```python
from build123d import *

# Parameters (mm, degrees)
SKETCH1_R           = 5
BOSS_EXTRUDE1_DEPTH = 5


with BuildPart() as part:
    # Sketch1 → Boss-Extrude1 (new body)
    with BuildSketch(Plane.XY):
        with BuildLine():
            Line((9.797958971, 5), (150.202041029, 5))
            ThreePointArc((150.202041029, 5), (152.091863394, 5.370899501), (153.70131209, 6.428571429))
            ThreePointArc((153.70131209, 6.428571429), (169, 0), (153.70131209, -6.428571429))
            ThreePointArc((153.70131209, -6.428571429), (152.091863394, -5.370899501), (150.202041029, -5))
            Line((150.202041029, -5), (9.797958971, -5))
            ThreePointArc((9.797958971, -5), (7.908136606, -5.370899501), (6.29868791, -6.428571429))
            ThreePointArc((6.29868791, -6.428571429), (-9, 0), (6.29868791, 6.428571429))
            ThreePointArc((6.29868791, 6.428571429), (7.908136606, 5.370899501), (9.797958971, 5))
        make_face()
        Circle(SKETCH1_R, mode=Mode.SUBTRACT)
        with Locations((160, 0)):
            Circle(SKETCH1_R, mode=Mode.SUBTRACT)
    extrude(amount=BOSS_EXTRUDE1_DEPTH)


solid = part.part
```
The listing builds one solid part. Answer for the finished solid, in the listing's coordinates (mm). A direction names the side the tool comes from. Round coordinates to 2 decimals unless told otherwise and drop trailing zeros. Loops run counter-clockwise (first coordinate to the right, second up) from the corner with the lowest first, then second, coordinate; pieces in that order, holes last.
Q1. For a pull along Y with two mould halves and no side action, classify faces 1 (the face through (7.93, -5.36, 2.46)), 2 (the face through (81, 0, 5)), 3 (the face through (-1.08, -4.88, 2.46)) as released by +Y, released by -Y, zero draft, split by the parting line, or undercut.
Q2. Which of the six approach directions +Z, -Z, +X, -X, +Y, -Y give full straight-line access (tool end or side, diameter ignored) to faces 4 (the face through (152.07, 5.36, 2.46)), 5 (the face through (81, -5, 2)), 6 (the face through (169, 0, 2))?
Q3. Section C-C, the plane y = 2.75 is taken. Determine the outline of the cut face in (x, z), then the cut area to 3 significant figures.
Q4. Section D-D, the plane x = 144.5 is taken. Determine the outline of the cut face in (y, z), then the cut area to 3 significant figures.
Q5. Given pin 1 Ø1.5 at (x, y) = (142.5, 6.5) entering from +Z; pin 2 Ø1.5 at (y, z) = (-1, 3) entering from +X; pin 3 Ø1.5 at (x, z) = (90, 1.5) entering from +Y; pin 4 Ø2 at (y, z) = (3, 1.5) entering from -X, each flat-ended and moving along its own axis, determine where each tip first touches the part or whether it passes through.
Q6. Section B-B, the plane z = 2.35 is taken. Determine the outline of the cut face in (x, y).
Q7. Section A-A, the plane x = 0 is taken. Determine the outline of the cut face in (y, z).
Q8. Find the intervals of material crossed by line 1 (Y direction, x = 160, z = 1.6); line 2 (X direction, y = 1.5, z = 3.4); line 3 (X direction, y = -2.75, z = 2.7), in increasing order.
Completed:
1. face 1: released by -Y
1. face 2: zero draft
1. face 3: undercut
2. face 4: +Z, -Z, +Y
2. face 5: +Z, -Z, -Y
2. face 6: +Z, -Z
3. outline: (-8.57, 0) - (-4.18, 0) - (-4.18, 5) - (-8.57, 5) - close; (4.18, 0) - (155.82, 0) - (155.82, 5) - (4.18, 5) - close; (164.18, 0) - (168.57, 0) - (168.57, 5) - (164.18, 5) - close
3. area: 802 mm2
4. outline: (-5, 0) - (5, 0) - (5, 5) - (-5, 5) - close
4. area: 50.0 mm2
5. pin 1: passes through
5. pin 2: stops at x = 169
5. pin 3: stops at y = 5
5. pin 4: stops at x = -8.77
6. outline: (6.3, -6.43) arc R5 cw to (9.8, -5) - (150.2, -5) arc R5 cw to (153.7, -6.43) arc R9 ccw (long way) to (153.7, 6.43) arc R5 cw to (150.2, 5) - (9.8, 5) arc R5 cw to (6.3, 6.43) arc R9 ccw (long way) to start; hole circle Ø10 at (0, 0); hole circle Ø10 at (160, 0)
7. outline: (-9, 0) - (-5, 0) - (-5, 5) - (-9, 5) - close; (5, 0) - (9, 0) - (9, 5) - (5, 5) - close
8. line 1: y = -9 to -5, 5 to 9
8. line 2: x = -8.87 to -4.77, 4.77 to 155.23, 164.77 to 168.87
8. line 3: x = -8.57 to -4.18, 4.18 to 155.82, 164.18 to 168.57
